Design review of the part built by this model. Coordinates are the model's own, in mm. A direction names the side the tool comes from. Coordinates: 2 decimals unless noted, no trailing zeros. Loops run counter-clockwise (first coordinate to the right, second up) from the corner with the lowest first, then second, coordinate; pieces in that order, holes last. Notation, with made-up numbers: (83, 29.25) -> (121, 29.25) arc R23 cw to (121, 64.25) -> close; hole circle Ø6 at (43, 77.5). An arc over 180 degrees is marked (long way). Use CSV: the item, a comma, the result in double quotes.
```python
from build123d import *

# Parameters (mm, degrees)
BOSS_EXTRUDE1_DEPTH = 5
SKETCH2_W           = 20
SKETCH2_H           = 160
CUT_EXTRUDE1_DEPTH  = 10


with BuildPart() as part:
    # Sketch1 → Boss-Extrude1 (new, symmetric)
    with BuildSketch(Plane.XY):
        with BuildLine():
            Line((-63.274211694, 196.041766301), (-20, 40))
            Line((-20, 40), (-20, 30))
            Line((-20, 30), (20, 30))
            Line((20, 30), (20, 40))
            Line((20, 40), (63.274211694, 196.041766301))
            ThreePointArc((63.274211694, 196.041766301), (0, 206), (-63.274211694, 196.041766301))
        make_face()
    extrude(amount=BOSS_EXTRUDE1_DEPTH, both=True)

    # Sketch2 → Cut-Extrude1 (cut)
    with BuildSketch(Plane.XY.offset(5)):
        with Locations((0, 30)):
            Rectangle(SKETCH2_W, SKETCH2_H)
    extrude(amount=-CUT_EXTRUDE1_DEPTH, mode=Mode.SUBTRACT)


solid = part.part
```
Item 1: Draft analysis for pull direction X (two halves, no side actions). For faces 1 (the face through (41.334, 116.929, 0.07)), 2 (the face through (-10, 69, 0)), 3 (the face through (-41.94, 119.11, 0.07)), state which applies: pulls with the +X half, pulls with the -X half, needs draft (parallel to the pull), parting line crosses it, or undercut.
Checked values:
face 1,"pulls with the +X half"
face 2,"undercut"
face 3,"pulls with the -X half"
Item 2: Add section A-A (z = -1.25). Give the boundary of the cut face in (x, y).
Checked values:
outline,"(-63.27, 196.04) -> (-20, 40) -> (-20, 30) -> (-10, 30) -> (-10, 110) -> (10, 110) -> (10, 30) -> (20, 30) -> (20, 40) -> (63.27, 196.04) arc R206 ccw to start"
Item 3: Add section C-C (x = -7). Give the boundary of the cut face in (y, z).
Checked values:
outline,"(110, -5) -> (205.88, -5) -> (205.88, 5) -> (110, 5) -> close"
Item 4: Machinability: for faces 4 (the face through (20, 35, 0)), 5 (the face through (-20, 35, 0)), 6 (the face through (0, 110, 0)), 7 (the face through (15, 30, 0)), which of the approach directions +Z, -Z, +X, -X, +Y, -Y give a long, thin tool a straight path to every point of the face, cutting with its end or side? Answer none if there is none.
Checked values:
face 4,"+Z, -Z, +X, -Y"
face 5,"+Z, -Z, -X, -Y"
face 6,"+Z, -Z, -Y"
face 7,"+Z, -Z, +X, -X, -Y"
Item 5: Add section B-B (y = 96.5). Give the boundary of the cut face in (x, z), then the cut area to 3 significant figures.
Checked values:
outline,"(-35.67, -5) -> (-10, -5) -> (-10, 5) -> (-35.67, 5) -> close; (10, -5) -> (35.67, -5) -> (35.67, 5) -> (10, 5) -> close"
area,"513 mm^2"
Item 6: Add section D-D (y = 143). Give the boundary of the cut face in (x, z).
Checked values:
outline,"(-48.56, -5) -> (48.56, -5) -> (48.56, 5) -> (-48.56, 5) -> close"
Item 7: To check wall thickness, follow line 1 along X through (y, z) = (94, -3.25); line 2 along X through (y, z) = (52.5, 2); line 3 along X through (y, z) = (134, -1.25). State the ranges of each line that lie inside material, in increasing order.
Checked values:
line 1,"-34.98 to -10, 10 to 34.98"
line 2,"-23.47 to -10, 10 to 23.47"
line 3,"-46.07 to 46.07"
Item 8: Clearance check with flat-ended pins moving along their axes: pin 1 (1 mm diameter, centred on x = -17.5, z = -4, fed in from +Y); pin 2 (3 mm diameter, centred on x = 4.5, z = -2.5, fed in from -Y); pin 3 (2 mm diameter, centred on y = 91, z = 1.5, fed in from +X). State where each tip first meets the part, or that it passes through.
Checked values:
pin 1,"y = 205.3"
pin 2,"y = 110"
pin 3,"x = 34.42"
